Verification items for the finished model (mm, model axes). Face numbers are marked on the shaded views. Give positions to 0.01 mm unless a question says otherwise; leave off trailing zeros. Order: outer loops, then holes, each group sorted by start corner. A loop starts at its lowest first (then second) coordinate and runs counter-clockwise, first axis right, second up.
(1) Sectioned sample at D-D on y = 225. Record the cut outline in (x, z), plus the area to 3 significant figures.
(2) Mould release check, pull along Y, two halves, no side actions. Record for the marked faces 1 and 2: pulls with the +Y half, pulls with the -Y half, needs draft (parallel to the pull), parting line crosses it, or undercut.
(3) Gauge pin test, flat ends, axial feed: pin 1 (8 mm diameter, centred on y = 227, z = 15.5, fed in from +X); pin 2 (1.5 mm diameter, centred on x = 216.5, z = 9, fed in from -Y); pin 3 (6 mm diameter, centred on x = 230, z = 9.5, fed in from +Y); pin 4 (4.5 mm diameter, centred on x = 330, z = 11, fed in from +Y). Record the tip position at first contact, or that the pin passes through.
(4) Sectioned sample at B-B on y = 121. Record the cut outline in (x, z).
(5) Scan lines: L1, parallel to X at y = 289.5, z = 6.5; L2, parallel to Y at x = 608.1, z = 11; L3, parallel to X at y = 1.35, z = 11. Record each from-to range of solid material in increasing order.
(6) Sectioned sample at C-C on x = 58. Record the cut outline in (y, z).
(7) Sectioned sample at A-A on y = 163. Record the cut outline in (x, z).
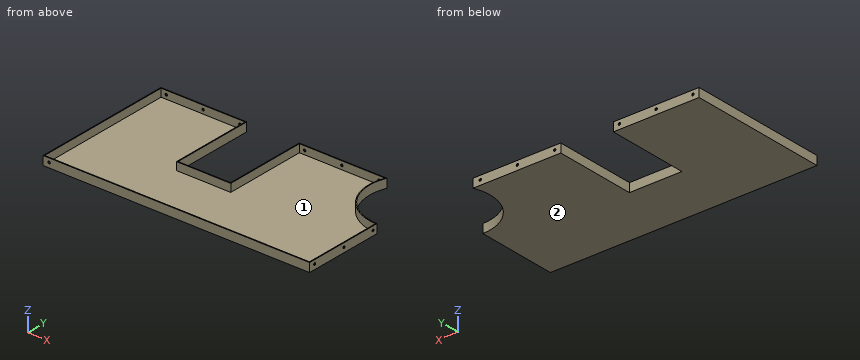
```python
from build123d import *

# Parameters (mm, degrees)
EXTRUDE_1_DEPTH          = 20
SHELL_1_T                = -2
CUT_EXTRUDE_1_DEPTH      = 338
CUT_EXTRUDE_1_DEPTH_BACK = 10
SKETCH_2_R               = 2.75
SKETCH_3_R               = 2.75
CUT_EXTRUDE_2_DEPTH      = 10
SKETCH_4_R               = 2.75
CUT_EXTRUDE_3_DEPTH      = 10


with BuildPart() as part:
    # 草图1 → 凸台-拉伸1 (new body)
    with BuildSketch(Plane.XY):
        with BuildLine():
            Line((0, 0), (609, 0))
            Line((609, 0), (609, 185))
            ThreePointArc((609, 185), (525.933761371, 229.322356372), (516.501351361, 323))
            Line((516.501351361, 323), (316, 323))
            Line((316, 323), (316, 135))
            Line((316, 135), (196, 135))
            Line((196, 135), (196, 323))
            Line((196, 323), (0, 323))
            Line((0, 323), (0, 0))
        make_face()
    extrude(amount=EXTRUDE_1_DEPTH)

    # 抽壳1
    shell_1_openings = [part.faces().sort_by_distance(p)[0] for p in [
        (304.5, 6.893547708, 20),
    ]]
    offset(amount=SHELL_1_T, openings=shell_1_openings, kind=Kind.INTERSECTION)

    # 草图2 → 切除-拉伸1 (cut, two sides: drawn at the far end of the back side and taken through both)
    with BuildSketch(Plane(origin=(0, 2, 0), x_dir=(1, 0, 0), z_dir=(0, 1, 0)).offset(-CUT_EXTRUDE_1_DEPTH_BACK)):
        with Locations(Location((14, -11, 0), (0, 0, 90))):
            Circle(SKETCH_2_R)
    extrude(amount=CUT_EXTRUDE_1_DEPTH + CUT_EXTRUDE_1_DEPTH_BACK, mode=Mode.SUBTRACT)

    # 草图3 → 切除-拉伸2 (cut)
    with BuildSketch(Plane.XZ.offset(-321)):
        with Locations(Location((98, 11, 0), (0, 0, 270))):
            Circle(SKETCH_3_R)
        with Locations(Location((182, 11, 0), (0, 0, 270))):
            Circle(SKETCH_3_R)
        with Locations(Location((330, 11, 0), (0, 0, 270))):
            Circle(SKETCH_3_R)
        with Locations(Location((415, 11, 0), (0, 0, 270))):
            Circle(SKETCH_3_R)
        with Locations(Location((500, 11, 0), (0, 0, 270))):
            Circle(SKETCH_3_R)
    extrude(amount=-CUT_EXTRUDE_2_DEPTH, mode=Mode.SUBTRACT)

    # 草图4 → 切除-拉伸3 (cut)
    with BuildSketch(Plane.ZY.offset(-607)):
        with Locations((11, 14)):
            Circle(SKETCH_4_R)
        with Locations((11, 94)):
            Circle(SKETCH_4_R)
        with Locations((11, 174)):
            Circle(SKETCH_4_R)
    extrude(amount=-CUT_EXTRUDE_3_DEPTH, mode=Mode.SUBTRACT)


solid = part.part
```
Ans:
1. outline: (0, 0) - (196, 0) - (196, 20) - (194, 20) - (194, 2) - (2, 2) - (2, 20) - (0, 20) - close; (316, 0) - (529, 0) - (529, 20) - (526.51, 20) - (526.51, 2) - (318, 2) - (318, 20) - (316, 20) - close
1. area: 971 mm2
2. face 1: undercut
2. face 2: needs draft
3. pin 1: stops at x = 530.54
3. pin 2: stops at y = 0
3. pin 3: stops at y = 135
3. pin 4: stops at y = 2
4. outline: (0, 0) - (609, 0) - (609, 20) - (607, 20) - (607, 2) - (2, 2) - (2, 20) - (0, 20) - close
5. L1: x = 0 to 2, 194 to 196, 316 to 318, 507.1 to 509.1
5. L2: y = 0 to 11.25, 16.75 to 91.25, 96.75 to 171.25, 176.75 to 185
5. L3: x = 0 to 11.25, 16.75 to 609
6. outline: (0, 0) - (323, 0) - (323, 20) - (321, 20) - (321, 2) - (2, 2) - (2, 20) - (0, 20) - close
7. outline: (0, 0) - (196, 0) - (196, 20) - (194, 20) - (194, 2) - (2, 2) - (2, 20) - (0, 20) - close; (316, 0) - (609, 0) - (609, 20) - (607, 20) - (607, 2) - (318, 2) - (318, 20) - (316, 20) - close
